Here's how the part is built. I have some questions about the finished solid (model axes, mm). Face numbers are marked on the shaded views. A direction names the side the tool comes from. Round coordinates to 2 decimals unless told otherwise and drop trailing zeros. Loops run counter-clockwise (first coordinate to the right, second up) from the corner with the lowest first, then second, coordinate; pieces in that order, holes last. Notation, with made-up numbers: M 3.5,8 L 15.5,8 A14 ccw 15.5,32 Z; hole C 6,44 d9. An arc over 180 degrees is marked long. Answer as a JSON object with one key per item and string values.
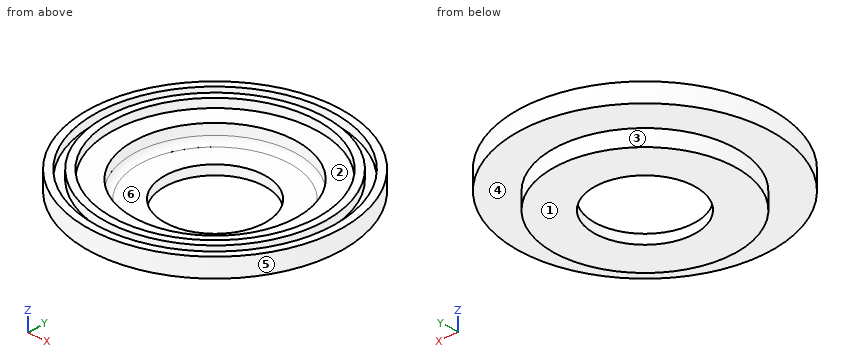
from build123d import *

# Parameters (mm, degrees)
FILLET1_R = 10


with BuildPart() as part:
    # Sketch1 → Revolve1 (revolve)
    with BuildSketch(Plane(origin=(0, 0, 0), x_dir=(0, 0, -1), z_dir=(1, 0, 0)), mode=Mode.PRIVATE) as revolve1_sk:
        Polygon((0, 164), (0, 176), (14, 176), (14, 190), (0, 190), (0, 202), (30, 202), (30, 145), (56, 145), (56, 80), (41, 80), (41, 130), (14, 130), (14, 164), align=None)
    revolve(revolve1_sk.sketch.rotate(Axis((0, 0, 0), (0, 0, -1)), 90), axis=Axis((0, 0, 0), (0, 0, -1)))

    # Fillet1
    fillet1_edges = [part.edges().sort_by_distance(p)[0] for p in [
        (-130, 0, -41),
    ]]
    fillet(fillet1_edges, radius=FILLET1_R)


solid = part.part
Item 1: If I drill on L1, parallel to Y at x = 0, z = -10; L2, parallel to Y at x = 27, z = -8; L3, parallel to X at y = -112.5, z = -3, over which ranges is the centre line in solid material (lowest first)? Write a range as from..to.
Solution:
{"L1": "y = -202..-190, -176..-164, 164..176, 190..202", "L2": "y = -200.19..-188.07, -173.92..-161.76, 161.76..173.92, 188.07..200.19", "L3": "x = -167.77..-153.11, -135.35..-119.33, 119.33..135.35, 153.11..167.77"}
Item 2: We'd pull the mould along Y, two halves only. Please class the marked faces 1, 2 and 3: +Y half, -Y half, draft (parallel to the pull), parting line (faces both ways), or undercut.
Solution:
{"face 1": "draft", "face 2": "undercut", "face 3": "parting line"}
Item 3: For P1, Ø1.5, axis at x = 108, y = -89.5, coming from the +Z side; P2, Ø1, axis at x = 32.5, z = -50.5, coming from the -Y side; P3, Ø5, axis at x = -107.5, z = -42, coming from the +Y side, each with a flat end and sliding along its axis, tell me the tip position at first contact or that it passes through.
Solution:
{"P1": "stops at z = -14", "P2": "stops at y = -141.42", "P3": "stops at y = 100"}
Item 4: I want a section at D-D on y = 135.5. List the corners of the cut face in (x, z) for me.
Solution:
{"outline": "M -149.81,-30 L -51.62,-30 L -51.62,-56 L 51.62,-56 L 51.62,-30 L 149.81,-30 L 149.81,0 L 133.19,0 L 133.19,-14 L 112.32,-14 L 112.32,0 L 92.39,0 L 92.39,-14 L -92.39,-14 L -92.39,0 L -112.32,0 L -112.32,-14 L -133.19,-14 L -133.19,0 L -149.81,0 Z"}
Item 5: For the marked faces 4, 5 and 6, which set-ups out of +Z, -Z, +X, -X, +Y, -Y let a thin tool reach every point of the face, with its end or its side?
Solution:
{"face 4": "-Z", "face 5": "+Z, -Z", "face 6": "+Z"}
Item 6: I want a section at C-C on z = -47.5. List the corners of the cut face in (x, y) for me, plus the area to 3 significant figures.
Solution:
{"outline": "C 0,0 d290; hole C 0,0 d160", "area": "45,900 mm2"}
